from build123d import *

# Parameters (mm, degrees)
SKETCH2_R               = 4.864
BOSS_EXTRUDE1_DEPTH     = 6
CUT_EXTRUDE1_DEPTH      = 25.460853079
CUT_EXTRUDE1_DEPTH_BACK = 25.460853079
SKETCH5_R               = 2.5
CUT_EXTRUDE2_DEPTH      = 20.244046698


with BuildPart() as part:
    # Sketch1 → Revolve1 (revolve)
    with BuildSketch(Plane.XY, mode=Mode.PRIVATE) as revolve1_sk:
        Polygon((0, 0), (0, 5.8), (0.5, 6.3), (6, 6.3), (6, 7), (12, 7), (12, 4.864), (21.5, 4.864), (22, 4.364), (22, 3.75), (6, 3.75), (6, 0), align=None)
    revolve(revolve1_sk.sketch.rotate(Axis((0, 0, 0), (1, 0, 0)), 90), axis=Axis((0, 0, 0), (1, 0, 0)))

    # Sketch2 → Boss-Extrude1 (add)
    with BuildSketch(Plane(origin=(12, 0, 0), x_dir=(0, 0, -1), z_dir=(1, 0, 0))):
        Polygon((8.082903769, 0), (4.041451884, 7), (-4.041451884, 7), (-8.082903769, 0), (-4.041451884, -7), (4.041451884, -7), align=None)
        with Locations(Location((0, 0, 0), (0, 0, 180))):
            Circle(SKETCH2_R, mode=Mode.SUBTRACT)
    extrude(amount=-BOSS_EXTRUDE1_DEPTH)

    # Sketch3 → Cut-Revolve1 (revolve, cut)
    with BuildSketch(Plane(origin=(0, 0, 0), x_dir=(1, 0, 0), z_dir=(0, 1, 0))):
        Polygon((10.917096231, 8.082903769), (12, 7), (12, 8.082903769), align=None)
        Polygon((6, 7), (7.082903769, 8.082903769), (6, 8.082903769), align=None)
    revolve(axis=Axis((0, 0, 0), (-1, 0, 0)), mode=Mode.SUBTRACT)

    # Sketch4 → Cut-Extrude1 (cut, two sides: drawn at the far end of the back side and taken through both)
    with BuildSketch(Plane.XY.offset(-CUT_EXTRUDE1_DEPTH_BACK)):
        Polygon((0, 2.886751346), (5, 0), (0, -2.886751346), align=None)
    extrude(amount=CUT_EXTRUDE1_DEPTH + CUT_EXTRUDE1_DEPTH_BACK, mode=Mode.SUBTRACT)

    # Sketch5 → Cut-Extrude2 (cut, through all)
    with BuildSketch(Plane(origin=(6, 0, 0), x_dir=(0, 0, -1), z_dir=(1, 0, 0))):
        Circle(SKETCH5_R)
    extrude(amount=-CUT_EXTRUDE2_DEPTH, mode=Mode.SUBTRACT)


solid = part.part
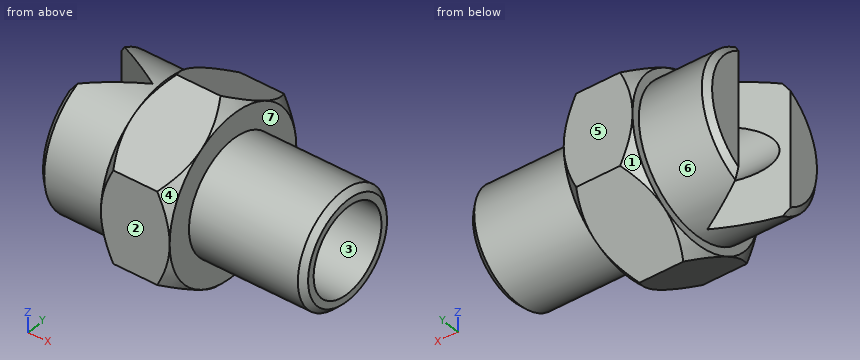
The listing builds one solid part. Answer for the finished solid, in the listing's coordinates (mm). Face numbers are marked on the shaded views. A direction names the side the tool comes from. Give positions to 0.01 mm unless a question says otherwise; leave off trailing zeros. Loops run counter-clockwise (first coordinate to the right, second up) from the corner with the lowest first, then second, coordinate; pieces in that order, holes last. Notation, with made-up numbers: (-1.5, 53.25) - (32.5, 53.25) arc R25 cw to (32.5, 85.25) - close; hole circle Ø8 at (77.5, 71.5). An arc over 180 degrees is marked (long way). Answer as a JSON object with one key per item and string values.
1. A cutting plane is placed at C-C (x = 2). Write down the section's boundary in (y, z).
Determined:
{"outline": "(-1.73, -6.06) - (-1.73, -1.8) arc R2.5 cw to (-1.73, 1.8) - (-1.73, 6.06) arc R6.3 ccw to start; (1.73, -6.06) arc R6.3 ccw to (1.73, 6.06) - (1.73, 1.8) arc R2.5 cw to (1.73, -1.8) - close"}
2. A cutting plane is placed at B-B (x = 8). Write down the section's boundary in (y, z).
Determined:
{"outline": "(-7, -4.04) - (0, -8.08) - (7, -4.04) - (7, 4.04) - (0, 8.08) - (-7, 4.04) - close; hole circle Ø7.5 at (0, 0)"}
3. For the marked faces 5, 6 and 7, determine the directions among +Z, -Z, +X, -X, +Y, -Y from which every point of the face is accessible in a straight line to the end or side of a thin tool.
Determined:
{"face 5": "+Z, -Z, +X, -X, +Y", "face 6": "-X", "face 7": "+X"}
4. Find the intervals of material crossed by L1, parallel to Y at x = 2.55, z = 0; L2, parallel to Y at x = 12.75, z = 0; L3, parallel to X at y = 5.75, z = 3.5, in increasing order. Write a range as [from, to].
Determined:
{"L1": "[-6.3, -2.5], [2.5, 6.3]", "L2": "[-4.86, -3.75], [3.75, 4.86]", "L3": "[6, 12]"}
5. Flat-ended cylindrical pins translate along their axes: pin 1 Ø4 at (x, z) = (19.5, 1.5) entering from -Y; pin 2 Ø5 at (x, z) = (3, -5) entering from +Y; pin 3 Ø1 at (x, z) = (7.5, -6.5) entering from -Y. Find the tip coordinate at first contact, or state that the pin passes through.
Determined:
{"pin 1": "y = -4.86", "pin 2": "y = 5.78", "pin 3": "y = -3.61"}
6. For a pull along Z with two mould halves and no side action, classify the marked faces 1, 2, 3 and 4 as pulls with the +Z half, pulls with the -Z half, needs draft (parallel to the pull), parting line crosses it, or undercut.
Determined:
{"face 1": "pulls with the -Z half", "face 2": "needs draft", "face 3": "undercut", "face 4": "pulls with the +Z half"}
7. A cutting plane is placed at D-D (x = 13.5). Write down the section's boundary in (y, z), then the cut area to 3 significant figures.
Determined:
{"outline": "circle Ø9.73 at (0, 0); hole circle Ø7.5 at (0, 0)", "area": "30.1 mm²"}
